The drawing under review shows one solid part. Ordinate dimensions are in mm from its lowest x, y, z. Round coordinates to 2 decimals unless told otherwise and drop trailing zeros. Loops run counter-clockwise (first coordinate to the right, second up) from the corner with the lowest first, then second, coordinate; pieces in that order, holes last. Notation, with made-up numbers: M 62.5,77 L 110.5,77 A20 cw 110.5,103 Z; hole C 87.5,87.5 d6. An arc over 180 degrees is marked long. Use a Markdown table: item, result.
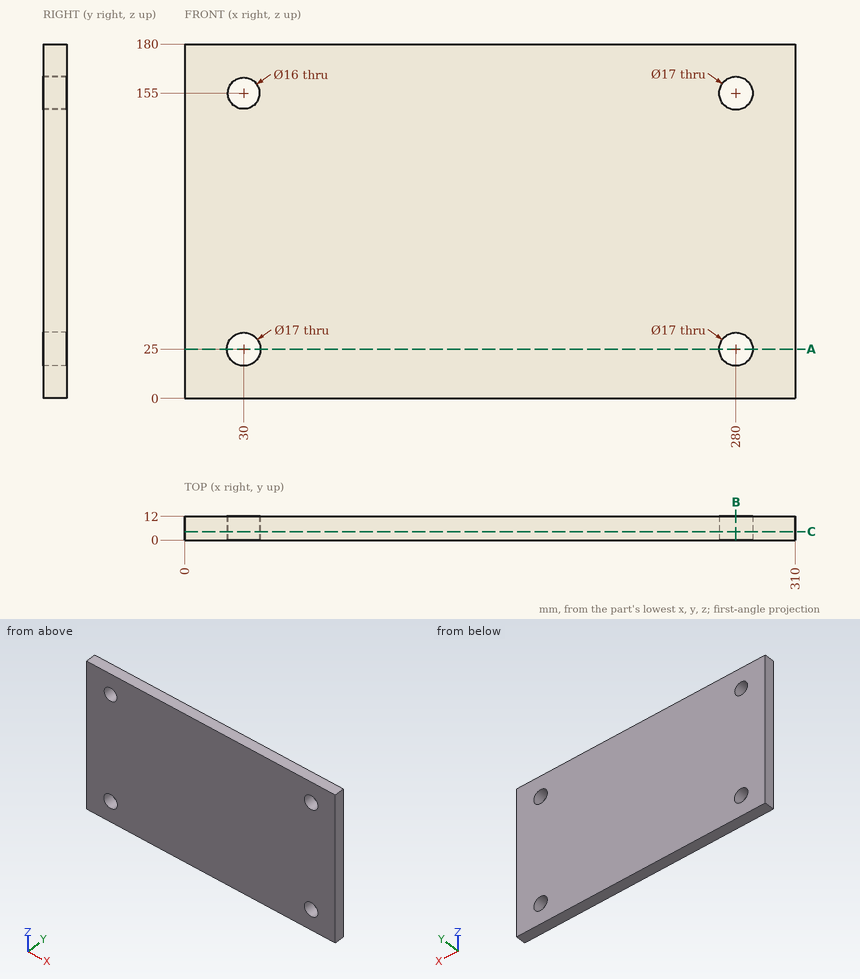
1. Wall thickness on line 1 along Z through (x, y) = (280, 9.25); line 2 along X through (y, z) = (4.25, 25); line 3 along X through (y, z) = (3, 155): over which ranges is each line inside the solid? List them lowest first. Write a range as from..to.
Check values:
| item | result |
|---|---|
| line 1 | z = 0..16.5, 33.5..146.5, 163.5..180 |
| line 2 | x = 0..21.5, 38.5..271.5, 288.5..310 |
| line 3 | x = 0..22, 38..271.5, 288.5..310 |
2. Take a section at C-C on y = 4.25. Give the boundary of the cut face in (x, z).
Check values:
| item | result |
|---|---|
| outline | M 0,0 L 310,0 L 310,180 L 0,180 Z; hole C 30,25 d17; hole C 30,155 d16; hole C 280,25 d17; hole C 280,155 d17 |
3. Take a section at A-A on z = 25. Give the boundary of the cut face in (x, y).
Check values:
| item | result |
|---|---|
| outline | M 0,0 L 21.5,0 L 21.5,12 L 0,12 Z; M 38.5,0 L 271.5,0 L 271.5,12 L 38.5,12 Z; M 288.5,0 L 310,0 L 310,12 L 288.5,12 Z |
4. Take a section at B-B on x = 280. Give the boundary of the cut face in (y, z).
Check values:
| item | result |
|---|---|
| outline | M 0,0 L 12,0 L 12,16.5 L 0,16.5 Z; M 0,33.5 L 12,33.5 L 12,146.5 L 0,146.5 Z; M 0,163.5 L 12,163.5 L 12,180 L 0,180 Z |
